Part print with two shaded views. Sizes in mm from the minimum x, y, z corner. A direction names the side the tool comes from. Round coordinates to 2 decimals unless told otherwise and drop trailing zeros. Loops run counter-clockwise (first coordinate to the right, second up) from the corner with the lowest first, then second, coordinate; pieces in that order, holes last.
(1) Tool access for the marked faces 1 and 2: list every direction of +Z, -Z, +X, -X, +Y, -Y with a clear straight run to the whole face (end or side of a thin tool).
(2) Cut at C-C on x = 120. List the corners of the cut face in (y, z).
(3) Mould opens along X. For the marked faces 3, 4 and 5 say: +X half, -X half, draft (parallel to the pull), parting line (faces both ways), or undercut.
(4) Cut at D-D on z = 31. List the corners of the cut face in (x, y).
(5) Cut at A-A on x = 90. List the corners of the cut face in (y, z).
(6) Cut at B-B on y = 87.5. List the corners of the cut face in (x, z) (1 decimal).
(7) Flat gauge pins, fed straight in: pin 1 (2 mm diameter, centred on x = 68.5, z = 12, fed in from -Y); pin 2 (6 mm diameter, centred on y = 23.5, z = 22, fed in from +X); pin 3 (8 mm diameter, centred on y = 30, z = 17, fed in from -X) (1 decimal); pin 4 (21.5 mm diameter, centred on x = 120, y = 141.96, fed in from +Z). Where does each tip first touch, or does it go through?
(8) Probe probe 1 along X at (y, z) = (89.5, 34) (1 decimal); probe 2 along Z at (x, y) = (106, 164.5). List the from-to ranges inside material, lowest first.
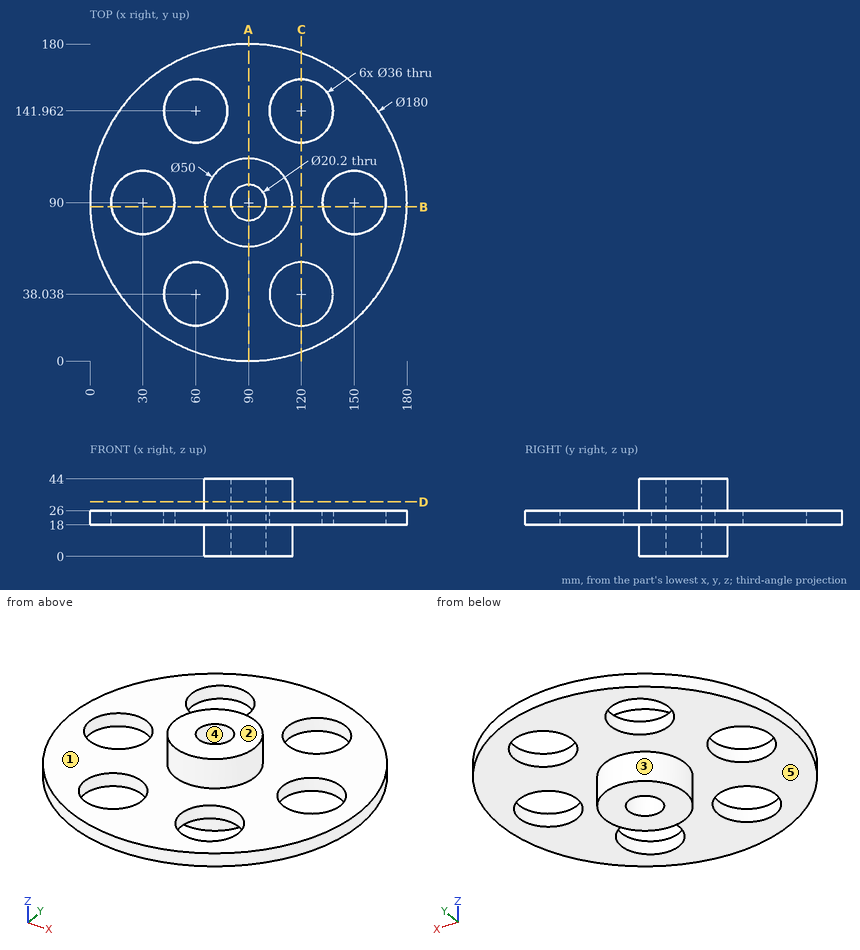
Final values:
1. face 1: +Z
1. face 2: +Z, +X, -X, +Y, -Y
2. outline: (5.15, 18) - (20.04, 18) - (20.04, 26) - (5.15, 26) - close; (56.04, 18) - (123.96, 18) - (123.96, 26) - (56.04, 26) - close; (159.96, 18) - (174.85, 18) - (174.85, 26) - (159.96, 26) - close
3. face 3: parting line
3. face 4: undercut
3. face 5: draft
4. outline: circle Ø50 at (90, 90); hole circle Ø20.2 at (90, 90)
5. outline: (0, 18) - (65, 18) - (65, 0) - (79.9, 0) - (79.9, 44) - (65, 44) - (65, 26) - (0, 26) - close; (100.1, 0) - (115, 0) - (115, 18) - (180, 18) - (180, 26) - (115, 26) - (115, 44) - (100.1, 44) - close
6. outline: (0, 18) - (12.2, 18) - (12.2, 26) - (0, 26) - close; (47.8, 18) - (65.1, 18) - (65.1, 0) - (80.2, 0) - (80.2, 44) - (65.1, 44) - (65.1, 26) - (47.8, 26) - close; (99.8, 0) - (114.9, 0) - (114.9, 18) - (132.2, 18) - (132.2, 26) - (114.9, 26) - (114.9, 44) - (99.8, 44) - close; (167.8, 18) - (180, 18) - (180, 26) - (167.8, 26) - close
7. pin 1: stops at y = 75.69
7. pin 2: stops at x = 153.78
7. pin 3: stops at x = 19.6
7. pin 4: passes through
8. probe 1: x = 65 to 79.9, 100.1 to 115
8. probe 2: z = 18 to 26
